The listing builds one solid part. Answer for the finished solid, in the listing's coordinates (mm). Face numbers are marked on the shaded views. A direction names the side the tool comes from. Coordinates: 2 decimals unless noted, no trailing zeros. Order: outer loops, then holes, each group sorted by start corner. A loop starts at its lowest first (then second) coordinate and runs counter-clockwise, first axis right, second up. Notation, with made-up numbers: (-23.5, -31.5) -> (30.5, -31.5) arc R29 cw to (30.5, -6.5) -> close; hole circle Ø1 at (47, 72). An arc over 180 degrees is marked (long way). One line per question, with ' | ' between items.
from build123d import *

# Parameters (mm, degrees)
BASE_PLATE_80X60X10_DEPTH      = 10
BASE_CORNER_CHAMFER_10_SIZE    = 10
SLOTTED_UPRIGHT_WALL_DEPTH     = 8
SIDE_BLOCK_SKETCH_W            = 17
SIDE_BLOCK_SKETCH_H            = 20
SIDE_BLOCK_25_DEPTH            = 8
SIDE_BLOCK_TOP_CHAMFER_10_SIZE = 10
HOLE_PAD_DEPTH                 = 5
PAD_HOLE_SKETCH_R              = 3.5
PAD_HOLE_7_DEPTH               = 87.746757864
PIVOT_LUG_SKETCH_R             = 5
PIVOT_LUG_DEPTH                = 15
LUG_ROOT_FILLET_R2_R           = 2
RELIEF_GROOVE_SKETCH_W         = 6
RELIEF_GROOVE_SKETCH_H         = 5
RELIEF_GROOVE_6X5_DEPTH        = 50


with BuildPart() as part:
    # Base Plate Sketch → Base Plate 80x60x10 (new body)
    with BuildSketch(Plane(origin=(0, 0, 0), x_dir=(1, 0, 0), z_dir=(0, 1, 0))):
        with BuildLine():
            Line((0, 0), (0, 30))
            Line((0, 30), (40, 30))
            Line((40, 30), (40, 15))
            ThreePointArc((40, 15), (45, 10), (50, 15))
            Line((50, 15), (50, 30))
            Line((50, 30), (80, 30))
            Line((80, 30), (80, -20))
            Line((80, -20), (60, -30))
            Line((60, -30), (0, -30))
            Line((0, -30), (0, 0))
        make_face()
    extrude(amount=BASE_PLATE_80X60X10_DEPTH)

    # Base Corner Chamfer 10
    base_corner_chamfer_10_edges = [part.edges().sort_by_distance(p)[0] for p in [
        (80, 5, -30),
    ]]
    chamfer(base_corner_chamfer_10_edges, length=BASE_CORNER_CHAMFER_10_SIZE)

    # Slotted Wall Sketch → Slotted Upright Wall (add)
    with BuildSketch(Plane.ZY):
        with BuildLine():
            Line((20, 30), (-30, 30))
            Line((-30, 30), (-30, 10))
            Line((-30, 10), (30, 10))
            Line((30, 10), (30, 20))
            ThreePointArc((30, 20), (27.071067812, 27.071067812), (20, 30))
        make_face()
        with BuildLine():
            Line((20, 16), (-5, 16))
            ThreePointArc((-5, 16), (-9, 20), (-5, 24))
            Line((-5, 24), (20, 24))
            ThreePointArc((20, 24), (24, 20), (20, 16))
        make_face(mode=Mode.SUBTRACT)
    extrude(amount=-SLOTTED_UPRIGHT_WALL_DEPTH)

    # Side Block Sketch → Side Block 25 (add)
    with BuildSketch(Plane(origin=(0, 0, -30), x_dir=(-1, 0, 0), z_dir=(0, 0, -1))):
        with Locations((-16.5, 20)):
            Rectangle(SIDE_BLOCK_SKETCH_W, SIDE_BLOCK_SKETCH_H)
    extrude(amount=-SIDE_BLOCK_25_DEPTH)

    # Side Block Top Chamfer 10
    side_block_top_chamfer_10_edges = [part.edges().sort_by_distance(p)[0] for p in [
        (25, 30, -26),
    ]]
    chamfer(side_block_top_chamfer_10_edges, length=SIDE_BLOCK_TOP_CHAMFER_10_SIZE)

    # Hole Pad Sketch → Hole Pad (add)
    with BuildSketch(Plane(origin=(0, 10, 0), x_dir=(1, 0, 0), z_dir=(0, 1, 0))):
        with BuildLine():
            Line((28, -18), (28, -30))
            Line((28, -30), (42, -30))
            Line((42, -30), (42, -18))
            ThreePointArc((42, -18), (35, -11), (28, -18))
        make_face()
    extrude(amount=HOLE_PAD_DEPTH)

    # Pad Hole Sketch → Pad Hole Ø7 (cut, through all)
    with BuildSketch(Plane(origin=(0, 15, 0), x_dir=(1, 0, 0), z_dir=(0, 1, 0))):
        with Locations(Location((35, -18, 0), (0, 0, 270))):
            Circle(PAD_HOLE_SKETCH_R)
    extrude(amount=-PAD_HOLE_7_DEPTH, mode=Mode.SUBTRACT)

    # Pivot Lug Sketch → Pivot Lug (add)
    with BuildSketch(Plane(origin=(80, 0, 0), x_dir=(0, 0, -1), z_dir=(1, 0, 0))):
        with BuildLine():
            Line((-9, 22), (-9, 10))
            Line((-9, 10), (9, 10))
            Line((9, 10), (9, 22))
            ThreePointArc((9, 22), (0, 31), (-9, 22))
        make_face()
        with Locations((0, 22)):
            Circle(PIVOT_LUG_SKETCH_R, mode=Mode.SUBTRACT)
    extrude(amount=-PIVOT_LUG_DEPTH)

    # Lug Root Fillet R2
    lug_root_fillet_r2_edges = [part.edges().sort_by_distance(p)[0] for p in [
        (72.5, 10, -9),
        (72.5, 10, 9),
        (35, 10, 11),
        (28, 10, 24),
        (42, 10, 24),
    ]]
    fillet(lug_root_fillet_r2_edges, radius=LUG_ROOT_FILLET_R2_R)

    # Relief Groove Sketch → Relief Groove 6x5 (cut)
    with BuildSketch(Plane(origin=(0, 0, -30), x_dir=(-1, 0, 0), z_dir=(0, 0, -1))):
        with Locations((-3, 2.5)):
            Rectangle(RELIEF_GROOVE_SKETCH_W, RELIEF_GROOVE_SKETCH_H)
    extrude(amount=-RELIEF_GROOVE_6X5_DEPTH, mode=Mode.SUBTRACT)


solid = part.part
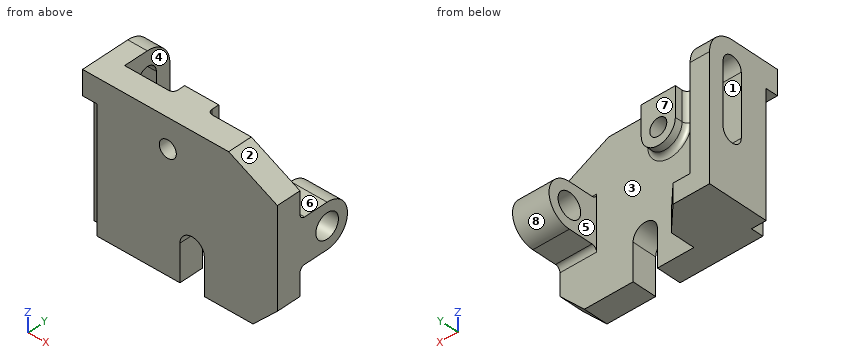
Item 1: Find the intervals of material crossed by L1, parallel to X at y = 29.5, z = -2; L2, parallel to Y at x = 73.5, z = 0; L3, parallel to X at y = 4.5, z = -18, in increasing order.
Computed values:
L1: x = 0 to 8, 65 to 80 | L2: y = 0 to 17, 27 to 31 | L3: x = 6 to 40, 50 to 80
Item 2: Section A-A, the plane y = 2 is taken. Give the vertices of the cut face in (x, z), plus the area to 3 significant figures.
Computed values:
outline: (0, 20) -> (6, 20) -> (6, -30) -> (40, -30) -> (40, -15) arc R5 cw to (50, -15) -> (50, -30) -> (70, -30) -> (80, -20) -> (80, 20) -> (60, 30) -> (0, 30) -> close; hole circle Ø7 at (35, 18) | area: 4,120 mm^2
Item 3: Section C-C, the plane x = 67.5 is taken. Give the vertices of the cut face in (y, z), plus the area to 3 significant figures.
Computed values:
outline: (0, -30) -> (10, -30) -> (10, -11) arc R2 cw to (12, -9) -> (22, -9) arc R9 ccw to (22, 9) -> (12, 9) arc R2 cw to (10, 11) -> (10, 26.25) -> (0, 26.25) -> close; hole circle Ø10 at (22, 0) | area: 829 mm^2
Item 4: For the marked faces 4, 5, 6, 7 and 8, determine the directions among +Z, -Z, +X, -X, +Y, -Y from which every point of the face is accessible in a straight line to the end or side of a thin tool.
Computed values:
face 4: +Z, +Y | face 5: +Z, -Z, +Y | face 6: +Z, +X, +Y | face 7: +Z, -Z, +X, +Y | face 8: +X, +Y
Item 5: Each of these flat-tipped pins is pushed along its axis until it touches: pin 1 Ø11.5 at (y, z) = (22, 0) entering from +X; pin 2 Ø5 at (x, z) = (2, -9) entering from -Y; pin 3 Ø9 at (x, z) = (2, 10.5) entering from +Y; pin 4 Ø2.5 at (y, z) = (13.5, 22) entering from +X. Where does it stop, or does it pass through?
Computed values:
pin 1: stops at x = 80 | pin 2: stops at y = 5 | pin 3: stops at y = 30 | pin 4: stops at x = 42
Item 6: Section D-D, the plane x = 35 is taken. Give the vertices of the cut face in (y, z).
Computed values:
outline: (0, -30) -> (10, -30) -> (10, 9) arc R2 cw to (12, 11) -> (15, 11) -> (15, 14.5) -> (0, 14.5) -> close; (0, 21.5) -> (15, 21.5) -> (15, 30) -> (0, 30) -> close
Item 7: Section B-B, the plane z = 0 is taken. Give the vertices of the cut face in (x, y).
Computed values:
outline: (0, 5) -> (6, 5) -> (6, 0) -> (80, 0) -> (80, 17) -> (65, 17) -> (65, 10) -> (8, 10) -> (8, 16) -> (0, 16) -> close; (0, 24) -> (8, 24) -> (8, 30) -> (0, 30) -> close; (65, 27) -> (80, 27) -> (80, 31) -> (65, 31) -> close
Item 8: Determine the mould class of the marked faces 1, 2 and 3 for opening direction X: pulls with the +X half, pulls with the -X half, needs draft (parallel to the pull), parting line crosses it, or undercut.
Computed values:
face 1: needs draft | face 2: pulls with the +X half | face 3: undercut
